from build123d import *

# Parameters (mm, degrees)
SKETCH_1_W          = 270
SKETCH_1_H          = 30
EXTRUDE_1_DEPTH     = 40
SKETCH_2_R          = 10
CUT_EXTRUDE_2_DEPTH = 30
SKETCH_5_W          = 30
SKETCH_5_H          = 40
CUT_EXTRUDE_4_DEPTH = 10
CUT_EXTRUDE_5_DEPTH = 144.961800489


with BuildPart() as part:
    # 草图1 → 凸台-拉伸1 (new body)
    with BuildSketch(Plane(origin=(0, 0, 0), x_dir=(1, 0, 0), z_dir=(0, 1, 0))):
        Rectangle(SKETCH_1_W, SKETCH_1_H)
    extrude(amount=EXTRUDE_1_DEPTH)

    # 草图2 → 切除-拉伸2 (cut)
    with BuildSketch(Plane(origin=(0, 40, 0), x_dir=(1, 0, 0), z_dir=(0, 1, 0))):
        with Locations(Location((70, 0, 0), (0, 0, 270))):
            Circle(SKETCH_2_R)
        with Locations(Location((-70, 0, 0), (0, 0, 90))):
            Circle(SKETCH_2_R)
    extrude(amount=-CUT_EXTRUDE_2_DEPTH, mode=Mode.SUBTRACT)

    # 草图5 → 切除-拉伸4 (cut)
    with BuildSketch(Plane(origin=(135, 0, 0), x_dir=(0, 0, -1), z_dir=(1, 0, 0))):
        with Locations((0, 20)):
            Rectangle(SKETCH_5_W, SKETCH_5_H)
    extrude(amount=-CUT_EXTRUDE_4_DEPTH, mode=Mode.SUBTRACT)

    # 草图6 → 切除-拉伸5 (cut, through all)
    with BuildSketch(Plane.XY.offset(15)):
        Polygon((125, 40), (85, 0), (125, 0), align=None)
    extrude(amount=-CUT_EXTRUDE_5_DEPTH, mode=Mode.SUBTRACT)


solid = part.part
Input: part model. Units: mm. Frame: model coordinates. A direction names the side the tool comes from. Coordinates: 2 decimals unless noted, no trailing zeros. Order: outer loops, then holes, each group sorted by start corner. A loop starts at its lowest first (then second) coordinate and runs counter-clockwise, first axis right, second up. Notation, with made-up numbers: M 60.25,-15.75 L 104.25,-15.75 A33 cw 104.25,22.25 Z; hole C 45,-13 d6. An arc over 180 degrees is marked long. Answer in a Markdown table with one row per item.
(1) Section query B-B, the plane z = 0. Output: boundary loops of the cut face in (x, y).
Numbers:
| item | result |
|---|---|
| outline | M -135,0 L 85,0 L 125,40 L 80,40 L 80,10 L 60,10 L 60,40 L -60,40 L -60,10 L -80,10 L -80,40 L -135,40 Z |
(2) Contact query for flat-ended pins moving along their axis: pin 1 Ø16 at (x, z) = (70, 0) entering from +Y; pin 2 Ø5 at (y, z) = (34.5, 11) entering from +X. Output: stop coordinate, or through.
Numbers:
| item | result |
|---|---|
| pin 1 | stops at y = 10 |
| pin 2 | stops at x = 122 |
(3) Draft query along Z for faces 1 (the cylindrical face through (79.915, 25.21, -1.302)), 2 (the flat face through (-7, 20, 15)), 3 (the flat face through (-27, 0, 0)). Return one class per face: pulls with the +Z half, pulls with the -Z half, needs draft (parallel to the pull), parting line crosses it, or undercut.
Numbers:
| item | result |
|---|---|
| face 1 | undercut |
| face 2 | pulls with the +Z half |
| face 3 | needs draft |
(4) Section query D-D, the plane x = 88. Output: boundary loops of the cut face in (y, z), plus the area to 3 significant figures.
Numbers:
| item | result |
|---|---|
| outline | M 3,-15 L 40,-15 L 40,15 L 3,15 Z |
| area | 1,110 mm^2 |
(5) Section query C-C, the plane y = 29. Output: boundary loops of the cut face in (x, z), plus the area to 3 significant figures.
Numbers:
| item | result |
|---|---|
| outline | M -135,-15 L 114,-15 L 114,15 L -135,15 Z; hole C -70,0 d20; hole C 70,0 d20 |
| area | 6,840 mm^2 |
(6) Section query A-A, the plane x = -70. Output: boundary loops of the cut face in (y, z), plus the area to 3 significant figures.
Numbers:
| item | result |
|---|---|
| outline | M 0,-15 L 40,-15 L 40,-10 L 10,-10 L 10,10 L 40,10 L 40,15 L 0,15 Z |
| area | 600 mm^2 |
(7) Access query for faces 4 (the flat face through (105, 20, 0)), 5 (the cylindrical face through (-79.915, 25.21, 1.302)). Directions: +Z, -Z, +X, -X, +Y, -Y. A direction counts if a zero-diameter tool reaches every point of the face in a straight line with its end or side. Return the directions, or none.
Numbers:
| item | result |
|---|---|
| face 4 | +Z, -Z, +X, -Y |
| face 5 | +Y |
(8) Material intervals for line 1 (X direction, y = 33, z = 0); line 2 (Z direction, x = -70, y = 21.75); line 3 (X direction, y = 22.25, z = 0), sorted ascending. Write a range as [from, to].
Numbers:
| item | result |
|---|---|
| line 1 | x = [-135, -80], [-60, 60], [80, 118] |
| line 2 | z = [-15, -10], [10, 15] |
| line 3 | x = [-135, -80], [-60, 60], [80, 107.25] |
